Design review of the part built by this model. Coordinates are the model's own, in mm. Give positions to 0.01 mm unless a question says otherwise; leave off trailing zeros. Loops run counter-clockwise (first coordinate to the right, second up) from the corner with the lowest first, then second, coordinate; pieces in that order, holes last. Notation, with made-up numbers: (-3.75, 25) - (35.25, 25) arc R23 cw to (35.25, 33) - close; hole circle Ø8 at (49.5, -0.5). An arc over 180 degrees is marked (long way). Put each result on its own line as item: value. Start each with the question number.
```python
from build123d import *

# Parameters (mm, degrees)
BOSS_EXTRUDE1_DEPTH = 0.6


with BuildPart() as part:
    # Sketch1 → Boss-Extrude1 (new body)
    with BuildSketch(Plane.XY):
        with BuildLine():
            Line((0.655924801, 2.722087922), (0.655924801, 5.162028968))
            Line((0.655924801, 5.162028968), (2.012866642, 5.162028968))
            Line((2.012866642, 5.162028968), (2.012866642, 3.223099112))
            ThreePointArc((2.012866642, 3.223099112), (-0.275338884, -3.790011675), (-1.525882777, 3.480184155))
            Line((-1.525882777, 3.480184155), (-1.525882777, 5.162028968))
            Line((-1.525882777, 5.162028968), (-0.363562636, 5.162028968))
            Line((-0.363562636, 5.162028968), (-0.363562636, 2.776296492))
            ThreePointArc((-0.363562636, 2.776296492), (-0.148672631, -2.796050151), (0.655924801, 2.722087922))
        make_face()
    extrude(amount=BOSS_EXTRUDE1_DEPTH)


solid = part.part
```
Item 1: Consider section C-C (x = 1.25). State the section outline as (y, z) points.
Item 2: Consider section A-A (y = 4.25). State the section outline as (x, z) points.
Item 3: For P1, Ø2, axis at x = -1, y = 1, coming from the +Z side, flat-tipped, find the tip position at first contact; note if it passes through.
Item 4: For L1, parallel to X at y = 0, z = 0.35; L2, parallel to Y at x = 0, z = 0.45; L3, parallel to X at y = -1.25, z = 0.4, list the stretches that pass through material, from the lowest coordinate up. Write a range as from..to.
Item 5: Consider section B-B (z = 0.2). State the section outline as (x, y) points.
Item 6: Consider section D-D (x = 0). State the section outline as (y, z) points, plus the area to 3 significant figures.
Geometry says:
1. outline: (-3.59, 0) - (-2.51, 0) - (-2.51, 0.6) - (-3.59, 0.6) - close; (2.51, 0) - (5.16, 0) - (5.16, 0.6) - (2.51, 0.6) - close
2. outline: (-1.53, 0) - (-0.36, 0) - (-0.36, 0.6) - (-1.53, 0.6) - close; (0.66, 0) - (2.01, 0) - (2.01, 0.6) - (0.66, 0.6) - close
3. P1: passes through
4. L1: x = -3.8..-2.8, 2.8..3.8
4. L2: y = -3.8..-2.8
4. L3: x = -3.59..-2.51, 2.51..3.59
5. outline: (-1.53, 3.48) arc R3.8 ccw (long way) to (2.01, 3.22) - (2.01, 5.16) - (0.66, 5.16) - (0.66, 2.72) arc R2.8 cw (long way) to (-0.36, 2.78) - (-0.36, 5.16) - (-1.53, 5.16) - close
6. outline: (-3.8, 0) - (-2.8, 0) - (-2.8, 0.6) - (-3.8, 0.6) - close
6. area: 0.600 mm2
